Verification items for the finished model (mm, model axes). Face numbers are marked on the shaded views. A direction names the side the tool comes from. Round coordinates to 2 decimals unless told otherwise and drop trailing zeros. Loops run counter-clockwise (first coordinate to the right, second up) from the corner with the lowest first, then second, coordinate; pieces in that order, holes last. Notation, with made-up numbers: (-8.75, 32) - (-2.75, 32) arc R23 cw to (-2.75, 67) - close; hole circle Ø8 at (3.25, 24). An arc over 180 degrees is marked (long way). Use CSV: the item, a comma, the result in double quotes.
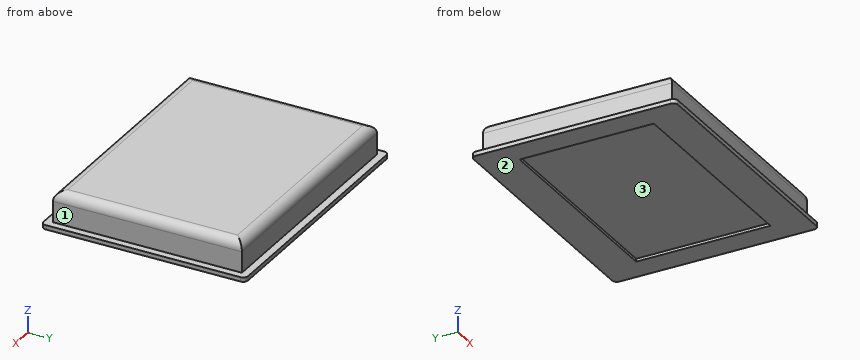
```python
from build123d import *

# Parameters (mm, degrees)
SKETCH_1_W          = 271
SKETCH_1_H          = 213
EXTRUDE_1_DEPTH     = 4.5
SKETCH_2_W          = 255
SKETCH_2_H          = 197
EXTRUDE_2_DEPTH     = 31.86
FILLET_1_R          = 10
FILLET_2_R          = 5
SKETCH_4_W          = 220
SKETCH_4_H          = 140
CUT_EXTRUDE_1_DEPTH = 3


with BuildPart() as part:
    # 草图1 → 凸台-拉伸1 (new body)
    with BuildSketch(Plane.XY):
        with Locations((135.5, -106.5)):
            Rectangle(SKETCH_1_W, SKETCH_1_H)
    extrude(amount=EXTRUDE_1_DEPTH)

    # 草图2 → 凸台-拉伸2 (add)
    with BuildSketch(Plane.XY.offset(4.5)):
        with Locations((135.5, -106.5)):
            Rectangle(SKETCH_2_W, SKETCH_2_H)
    extrude(amount=EXTRUDE_2_DEPTH)

    # 圆角1
    fillet_1_edges = [part.edges().sort_by_distance(p)[0] for p in [
        (263, -106.5, 36.36),
        (135.5, -8, 36.36),
        (8, -106.5, 36.36),
        (135.5, -205, 36.36),
    ]]
    fillet(fillet_1_edges, radius=FILLET_1_R)

    # 圆角2
    fillet_2_edges = [part.edges().sort_by_distance(p)[0] for p in [
        (0, 0, 2.25),
        (271, 0, 2.25),
        (271, -213, 2.25),
        (0, -213, 2.25),
    ]]
    fillet(fillet_2_edges, radius=FILLET_2_R)

    # 草图4 → 切除-拉伸1 (cut)
    with BuildSketch(Plane(origin=(0, 0, 0), x_dir=(-1, 0, 0), z_dir=(0, 0, -1))):
        with Locations((-135.5, -106.5)):
            Rectangle(SKETCH_4_W, SKETCH_4_H)
    extrude(amount=-CUT_EXTRUDE_1_DEPTH, mode=Mode.SUBTRACT)


solid = part.part
```
1) Cross-section at B-B, the plane x = 225. Record the cut outline in (y, z).
Returned:
outline,"(-213, 0) - (-176.5, 0) - (-176.5, 3) - (-36.5, 3) - (-36.5, 0) - (0, 0) - (0, 4.5) - (-8, 4.5) - (-8, 26.36) arc R10 ccw to (-18, 36.36) - (-195, 36.36) arc R10 ccw to (-205, 26.36) - (-205, 4.5) - (-213, 4.5) - close"
2) Cross-section at D-D, the plane y = -32.5. Record the cut outline in (x, z).
Returned:
outline,"(0, 0) - (271, 0) - (271, 4.5) - (263, 4.5) - (263, 26.36) arc R10 ccw to (253, 36.36) - (18, 36.36) arc R10 ccw to (8, 26.36) - (8, 4.5) - (0, 4.5) - close"
3) Gauge pin test, flat ends, axial feed: pin 1 Ø4 at (x, y) = (146.5, -116.5) entering from -Z; pin 2 Ø1 at (x, z) = (112, 23.5) entering from +Y; pin 3 Ø17.5 at (y, z) = (-135.5, 18.5) entering from -X. Record the tip position at first contact, or that the pin passes through.
Returned:
pin 1,"stops at z = 3"
pin 2,"stops at y = -8"
pin 3,"stops at x = 8"
4) Cross-section at C-C, the plane z = 17. Record the cut outline in (x, y), then the cut area to 3 significant figures.
Returned:
outline,"(8, -205) - (263, -205) - (263, -8) - (8, -8) - close"
area,"50,200 mm²"
5) Thickness scan on probe 1 along Z at (x, y) = (240.5, -116); probe 2 along Y at (x, z) = (175.5, 21.5); probe 3 along X at (y, z) = (-63, 22.5). Record the ranges inside material, lowest first. Write a range as [from, to].
Returned:
probe 1,"z = [3, 36.36]"
probe 2,"y = [-205, -8]"
probe 3,"x = [8, 263]"
6) Access from +Z, -Z, +X, -X, +Y, -Y to the whole of each face (thin tool, end or side, straight path). Record for the marked faces 1, 2 and 3.
Returned:
face 1,"+Z, +X, +Y, -Y"
face 2,"-Z, +X, -X, +Y, -Y"
face 3,"-Z"
7) Cross-section at A-A, the plane y = -86. Record the cut outline in (x, z).
Returned:
outline,"(0, 0) - (25.5, 0) - (25.5, 3) - (245.5, 3) - (245.5, 0) - (271, 0) - (271, 4.5) - (263, 4.5) - (263, 26.36) arc R10 ccw to (253, 36.36) - (18, 36.36) arc R10 ccw to (8, 26.36) - (8, 4.5) - (0, 4.5) - close"
